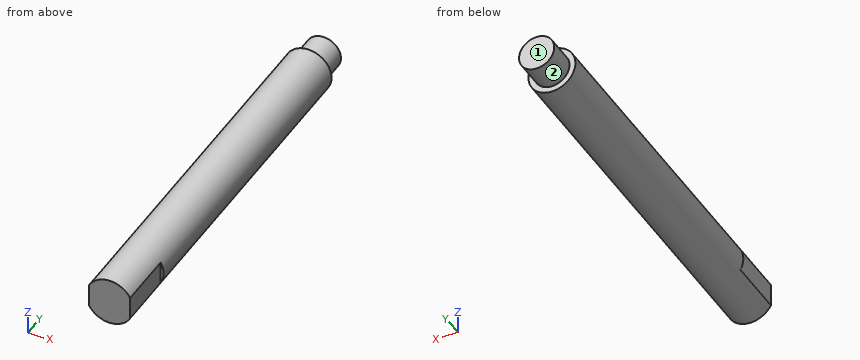
from build123d import *

# Parameters (mm, degrees)
SKETCH1_R           = 8
BOSS_EXTRUDE1_DEPTH = 130
SKETCH4_R           = 6
BOSS_EXTRUDE2_DEPTH = 10
SKETCH5_W           = 13.236787349
SKETCH5_H           = 35.235955056
SKETCH5_W_2         = 13.423220974
SKETCH5_H_2         = 24.946317104
CUT_EXTRUDE1_DEPTH  = 5


with BuildPart() as part:
    # Sketch1 → Boss-Extrude1 (new body)
    with BuildSketch(Plane(origin=(0, 0, 0), x_dir=(1, 0, 0), z_dir=(0, 1, 0))):
        with Locations(Location((0, 0, 0), (0, 0, 270))):
            Circle(SKETCH1_R)
    extrude(amount=BOSS_EXTRUDE1_DEPTH)

    # Sketch4 → Boss-Extrude2 (add)
    with BuildSketch(Plane(origin=(0, 130, 0), x_dir=(1, 0, 0), z_dir=(0, 1, 0))):
        with Locations(Location((0, 0, 0), (0, 0, 270))):
            Circle(SKETCH4_R)
    extrude(amount=BOSS_EXTRUDE2_DEPTH)

    # Sketch5 → Cut-Extrude1 (cut, symmetric)
    with BuildSketch(Plane.XY):
        with Locations((-13.618393675, 2.382022472)):
            Rectangle(SKETCH5_W, SKETCH5_H)
        with Locations((13.711610487, 7.526841448)):
            Rectangle(SKETCH5_W_2, SKETCH5_H_2)
    extrude(amount=CUT_EXTRUDE1_DEPTH, both=True, mode=Mode.SUBTRACT)


solid = part.part
Geometry: final body of the model. Coordinates: model frame, mm. Face numbers are marked on the shaded views. A direction names the side the tool comes from. Round coordinates to 2 decimals unless told otherwise and drop trailing zeros. Loops run counter-clockwise (first coordinate to the right, second up) from the corner with the lowest first, then second, coordinate; pieces in that order, holes last. Notation, with made-up numbers: (89, 81) - (145, 81) arc R25 ccw to (145, 98) - close; hole circle Ø3 at (-28.5, -34.5). An arc over 180 degrees is marked (long way). Write each question's results on one line, items separated by ' | '. Start each with the question number.
1) Cut plane B-B on z = 0. Return loops of the section in (x, y), then the cut area to 3 significant figures.
2) Access query for the marked faces 1 and 2. Directions: +Z, -Z, +X, -X, +Y, -Y. A direction counts if a zero-diameter tool reaches every point of the face in a straight line with its end or side. Return the directions, or none.
3) Cut plane A-A on x = 0. Return loops of the section in (y, z), then the cut area to 3 significant figures.
4) Line query: probe 1 along Z at (x, y) = (7, 85); probe 2 along X at (y, z) = (82, -0.25). Output: solid intervals per line, ascending. Write a range as [from, to].
5) Cut plane C-C on y = 48.5. Return loops of the section in (x, z).
6) First-contact query: P1, Ø1.5, axis at y = 34, z = -0.5, coming from the -X side; P2, Ø1, axis at y = 87, z = -3.5, coming from the -X side; P3, Ø0.8, axis at x = 7.5, z = 1, coming from the -Y side; P4, Ø3, axis at x = 2, y = 126, coming from the +Z side. Flat tips, straight axial feed; report the tip coordinate or a pass-through.
Verdict:
1) outline: (-8, 20) - (-7, 20) - (-7, 0) - (7, 0) - (7, 20) - (8, 20) - (8, 130) - (6, 130) - (6, 140) - (-6, 140) - (-6, 130) - (-8, 130) - close | area: 2,160 mm2
2) face 1: +Z, -Z, +X, -X, +Y | face 2: +Y
3) outline: (0, -8) - (130, -8) - (130, -6) - (140, -6) - (140, 6) - (130, 6) - (130, 8) - (0, 8) - close | area: 2,200 mm2
4) probe 1: z = [-3.87, 3.87] | probe 2: x = [-8, 8]
5) outline: circle Ø16 at (0, 0)
6) P1: stops at x = -8 | P2: stops at x = -7.42 | P3: stops at y = 20 | P4: stops at z = 7.98
